from build123d import *


with BuildPart() as part:
    # 草图1 → 旋转1 (revolve)
    with BuildSketch(Plane.XY, mode=Mode.PRIVATE) as revolve_1_sk:
        Polygon((-37.5, 0), (-37.5, 40), (-36.5, 40), (-36.5, 74.5), (-39, 74.5), (-39, 76), (-17.5, 76), (-12.5, 76), (-12.5, 51), (-17.5, 51), (-17.5, 36), (-30, 36), (-30, 33), (-32.5, 33), (-32.5, 0), align=None)
    revolve(revolve_1_sk.sketch.rotate(Axis((0, 0, 0), (0, 1, 0)), 270), axis=Axis((0, 0, 0), (0, 1, 0)))


solid = part.part
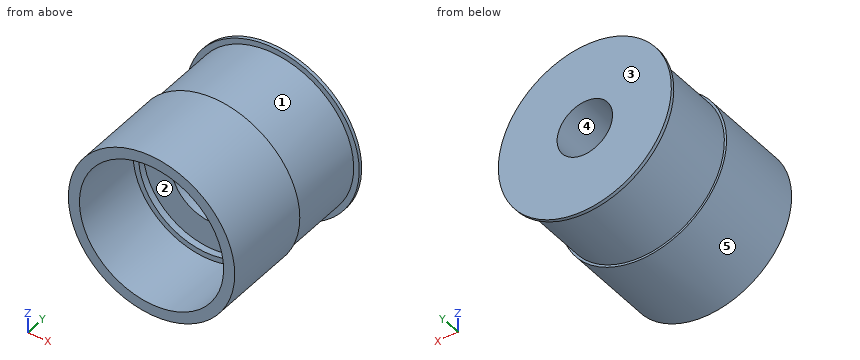
Work out the finished part from the listing and answer in its coordinate system (mm). Face numbers are marked on the shaded views. A direction names the side the tool comes from. Give positions to 0.01 mm unless a question says otherwise; leave off trailing zeros. Order: outer loops, then holes, each group sorted by start corner. A loop starts at its lowest first (then second) coordinate and runs counter-clockwise, first axis right, second up. Notation, with made-up numbers: (-9.75, 34.25) - (19.25, 34.25) arc R15 ccw to (19.25, 50.25) - close; hole circle Ø7 at (-10, 34.25). An arc over 180 degrees is marked (long way). Answer as CSV lines item,"result". Start each with the question number.
Q1. The part is cut by section C-C (y = 38.5). Write down the section's boundary in (x, z).
Q2. The part is cut by section A-A (z = 0). Write down the section's boundary in (x, y).
Q3. Given pin 1 Ø17.5 at (x, z) = (-2.5, -3.5) entering from -Y; pin 2 Ø6 at (y, z) = (56, -17.5) entering from -X; pin 3 Ø3 at (y, z) = (31.5, -23) entering from +X, each flat-ended and moving along its own axis, determine where each tip first touches the part or whether it passes through.
Q4. For the marked faces 4 and 5, determine the directions among +Z, -Z, +X, -X, +Y, -Y from which every point of the face is accessible in a straight line to the end or side of a thin tool.
Q5. Find the intervals of material crossed by L1, parallel to X at y = 34, z = 0; L2, parallel to X at y = 62, z = 0; L3, parallel to Y at x = 17.5, z = -7.5, in increasing order. Write a range as [from, to].
Q6. The mould has two halves that part along Z. Classify the marked faces 1, 2 and 3: +Z half, -Z half, draft (parallel to the pull), parting line (faces both ways), or undercut.
Q7. The part is cut by section D-D (x = -19). Write down the section's boundary in (y, z), then the cut area to 3 significant figures.
Q8. The part is cut by section B-B (x = 0). Write down the section's boundary in (y, z).
Check result:
1,outline,"circle Ø75 at (0, 0); hole circle Ø35 at (0, 0)"
2,outline,"(-39, 74.5) - (-36.5, 74.5) - (-36.5, 40) - (-37.5, 40) - (-37.5, 0) - (-32.5, 0) - (-32.5, 33) - (-30, 33) - (-30, 36) - (-17.5, 36) - (-17.5, 51) - (-12.5, 51) - (-12.5, 76) - (-39, 76) - close; (12.5, 51) - (17.5, 51) - (17.5, 36) - (30, 36) - (30, 33) - (32.5, 33) - (32.5, 0) - (37.5, 0) - (37.5, 40) - (36.5, 40) - (36.5, 74.5) - (39, 74.5) - (39, 76) - (12.5, 76) - close"
3,pin 1,"stops at y = 51"
3,pin 2,"stops at x = -33.5"
3,pin 3,"stops at x = 30.72"
4,face 4,"+Y, -Y"
4,face 5,"-Y"
5,L1,"x = [-37.5, -30], [30, 37.5]"
5,L2,"x = [-36.5, -12.5], [12.5, 36.5]"
5,L3,"y = [36, 76]"
6,face 1,"parting line"
6,face 2,"undercut"
6,face 3,"draft"
7,outline,"(0, -32.33) - (40, -32.33) - (40, -31.16) - (74.5, -31.16) - (74.5, -34.06) - (76, -34.06) - (76, 34.06) - (74.5, 34.06) - (74.5, 31.16) - (40, 31.16) - (40, 32.33) - (0, 32.33) - (0, 26.37) - (33, 26.37) - (33, 23.22) - (36, 23.22) - (36, -23.22) - (33, -23.22) - (33, -26.37) - (0, -26.37) - close"
7,area,"2,960 mm²"
8,outline,"(0, -37.5) - (40, -37.5) - (40, -36.5) - (74.5, -36.5) - (74.5, -39) - (76, -39) - (76, -12.5) - (51, -12.5) - (51, -17.5) - (36, -17.5) - (36, -30) - (33, -30) - (33, -32.5) - (0, -32.5) - close; (0, 32.5) - (33, 32.5) - (33, 30) - (36, 30) - (36, 17.5) - (51, 17.5) - (51, 12.5) - (76, 12.5) - (76, 39) - (74.5, 39) - (74.5, 36.5) - (40, 36.5) - (40, 37.5) - (0, 37.5) - close"
